The figure shows three views and two pictorial views of one solid part (mm, origin at its lowest corner). Answer the questions. Coordinates: 2 decimals unless noted, no trailing zeros. Write each loop counter-clockwise with the first axis right and the second up, starting at its lowest first coordinate (ties: lowest second). Pieces come first, ordered by that corner, then holes.
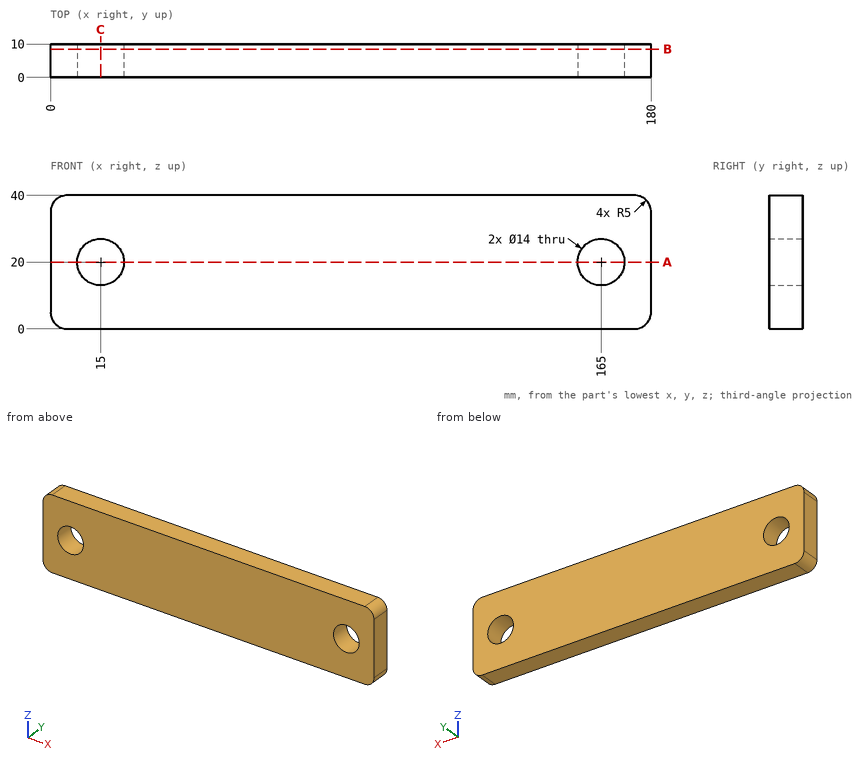
1. Section A-A on z = 20 is taken. Give the vertices of the cut face in (x, y).
Results found:
outline: (0, 0) - (8, 0) - (8, 10) - (0, 10) - close; (22, 0) - (158, 0) - (158, 10) - (22, 10) - close; (172, 0) - (180, 0) - (180, 10) - (172, 10) - close
2. Section B-B on y = 8.5 is taken. Give the vertices of the cut face in (x, z), then the cut area to 3 significant figures.
Results found:
outline: (0, 5) arc R5 ccw to (5, 0) - (175, 0) arc R5 ccw to (180, 5) - (180, 35) arc R5 ccw to (175, 40) - (5, 40) arc R5 ccw to (0, 35) - close; hole circle Ø14 at (15, 20); hole circle Ø14 at (165, 20)
area: 6,870 mm2
3. Find the intervals of material crossed by L1, parallel to X at y = 7.5, z = 20; L2, parallel to Z at x = 165, y = 6.25; L3, parallel to X at y = 3, z = 19, in increasing order.
Results found:
L1: x = 0 to 8, 22 to 158, 172 to 180
L2: z = 0 to 13, 27 to 40
L3: x = 0 to 8.07, 21.93 to 158.07, 171.93 to 180
4. Section C-C on x = 15 is taken. Give the vertices of the cut face in (y, z).
Results found:
outline: (0, 0) - (10, 0) - (10, 13) - (0, 13) - close; (0, 27) - (10, 27) - (10, 40) - (0, 40) - close
